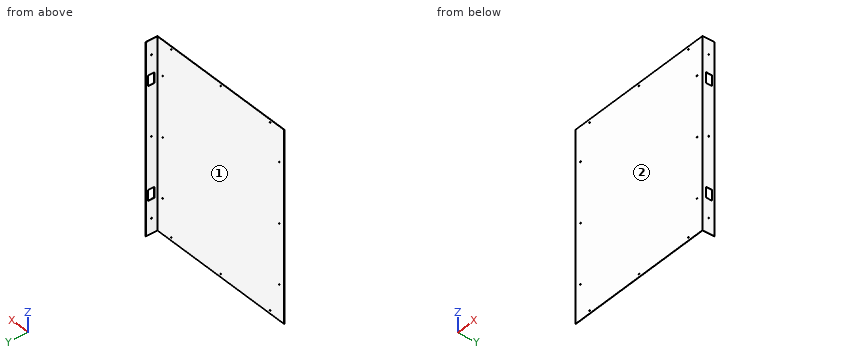
```python
from build123d import *

# Parameters (mm, degrees)
BOSS_EXTRUDE1_DEPTH = 950
SKETCH2_R           = 2.5
SKETCH2_W           = 53
SKETCH2_H           = 31
CUT_EXTRUDE1_DEPTH  = 1356.5
SKETCH3_R           = 2.5
CUT_EXTRUDE2_DEPTH  = 1.5
SKETCH4_W           = 1.5
SKETCH4_H           = 950
CUT_EXTRUDE3_DEPTH  = 58.5


with BuildPart() as part:
    # Sketch1 → Boss-Extrude1 (new body)
    with BuildSketch(Plane.XY):
        Polygon((0, 0), (0, -60), (770, -60), (770, 0), (768.5, 0), (768.5, -58.5), (1.5, -58.5), (1.5, 0), align=None)
    extrude(amount=BOSS_EXTRUDE1_DEPTH)

    # Sketch2 → Cut-Extrude1 (cut)
    with BuildSketch(Plane(origin=(770, 0, 0), x_dir=(0, 0, -1), z_dir=(1, 0, 0))):
        with Locations(Location((-75, -28.5, 0), (0, 0, 270))):
            Circle(SKETCH2_R)
        with Locations(Location((-475, -28.5, 0), (0, 0, 270))):
            Circle(SKETCH2_R)
        with Locations(Location((-875, -28.5, 0), (0, 0, 270))):
            Circle(SKETCH2_R)
        with Locations((-194.5, -27.5)):
            Rectangle(SKETCH2_W, SKETCH2_H)
        with Locations((-755.5, -27.5)):
            Rectangle(SKETCH2_W, SKETCH2_H)
    extrude(amount=-CUT_EXTRUDE1_DEPTH, mode=Mode.SUBTRACT)

    # Sketch3 → Cut-Extrude2 (cut)
    with BuildSketch(Plane.XZ.offset(60)):
        with Locations(Location((737, 475, 0), (0, 0, 270))):
            Circle(SKETCH3_R)
        with Locations(Location((737, 775, 0), (0, 0, 270))):
            Circle(SKETCH3_R)
        with Locations(Location((737, 175, 0), (0, 0, 270))):
            Circle(SKETCH3_R)
        with Locations(Location((30, 775, 0), (0, 0, 270))):
            Circle(SKETCH3_R)
        with Locations(Location((30, 475, 0), (0, 0, 270))):
            Circle(SKETCH3_R)
        with Locations(Location((30, 175, 0), (0, 0, 270))):
            Circle(SKETCH3_R)
        with Locations(Location((385, 935, 0), (0, 0, 270))):
            Circle(SKETCH3_R)
        with Locations(Location((685, 935, 0), (0, 0, 270))):
            Circle(SKETCH3_R)
        with Locations(Location((85, 935, 0), (0, 0, 270))):
            Circle(SKETCH3_R)
        with Locations(Location((85, 15, 0), (0, 0, 90))):
            Circle(SKETCH3_R)
        with Locations(Location((685, 15, 0), (0, 0, 90))):
            Circle(SKETCH3_R)
        with Locations(Location((385, 15, 0), (0, 0, 90))):
            Circle(SKETCH3_R)
    extrude(amount=-CUT_EXTRUDE2_DEPTH, mode=Mode.SUBTRACT)

    # Sketch4 → Cut-Extrude3 (cut)
    with BuildSketch(Plane(origin=(0, 0, 0), x_dir=(1, 0, 0), z_dir=(0, 1, 0))):
        with Locations((0.75, -475)):
            Rectangle(SKETCH4_W, SKETCH4_H)
    extrude(amount=-CUT_EXTRUDE3_DEPTH, mode=Mode.SUBTRACT)


solid = part.part
```
Model file for the job. Use its own axes, mm. Face numbers are marked on the shaded views. A direction names the side the tool comes from. Give positions to 0.01 mm unless a question says otherwise; leave off trailing zeros. Order: outer loops, then holes, each group sorted by start corner. A loop starts at its lowest first (then second) coordinate and runs counter-clockwise, first axis right, second up.
1) Saw through at B-B, the plane x = 569.5. Write the cut outline in (y, z).
2) 3-axis set-ups, long thin cutter, end or side, ignore diameter. For the marked faces 1 and 2: which of +Z, -Z, +X, -X, +Y, -Y reach the whole face in a straight line?
3) Pin check, flat tips, straight feed: pin 1 (1.6 mm diameter, centred on x = 769, y = -31, fed in from -Z); pin 2 (8 mm diameter, centred on y = -28.5, z = 75, fed in from -X); pin 3 (8 mm diameter, centred on x = 247, z = 537.5, fed in from +Y). Stop position of each tip, or through.
4) Saw through at A-A, the plane z = 504. Write the cut outline in (x, y).
5) Wall check: probe 1 along X at (y, z) = (-59.7, 15); probe 2 along Z at (x, y) = (685, -59); probe 3 along Z at (x, y) = (737, -59.7). Give the ranges that are in metal, low to high.
Computed:
1. outline: (-60, 0) - (-58.5, 0) - (-58.5, 950) - (-60, 950) - close
2. face 1: +Z, -Z, -X, +Y
2. face 2: +Z, -Z, +X, -X, -Y
3. pin 1: stops at z = 0
3. pin 2: stops at x = 768.5
3. pin 3: stops at y = -58.5
4. outline: (0, -60) - (770, -60) - (770, 0) - (768.5, 0) - (768.5, -58.5) - (0, -58.5) - close
5. probe 1: x = 0 to 82.5, 87.5 to 382.5, 387.5 to 682.5, 687.5 to 770
5. probe 2: z = 0 to 12.5, 17.5 to 932.5, 937.5 to 950
5. probe 3: z = 0 to 172.5, 177.5 to 472.5, 477.5 to 772.5, 777.5 to 950
